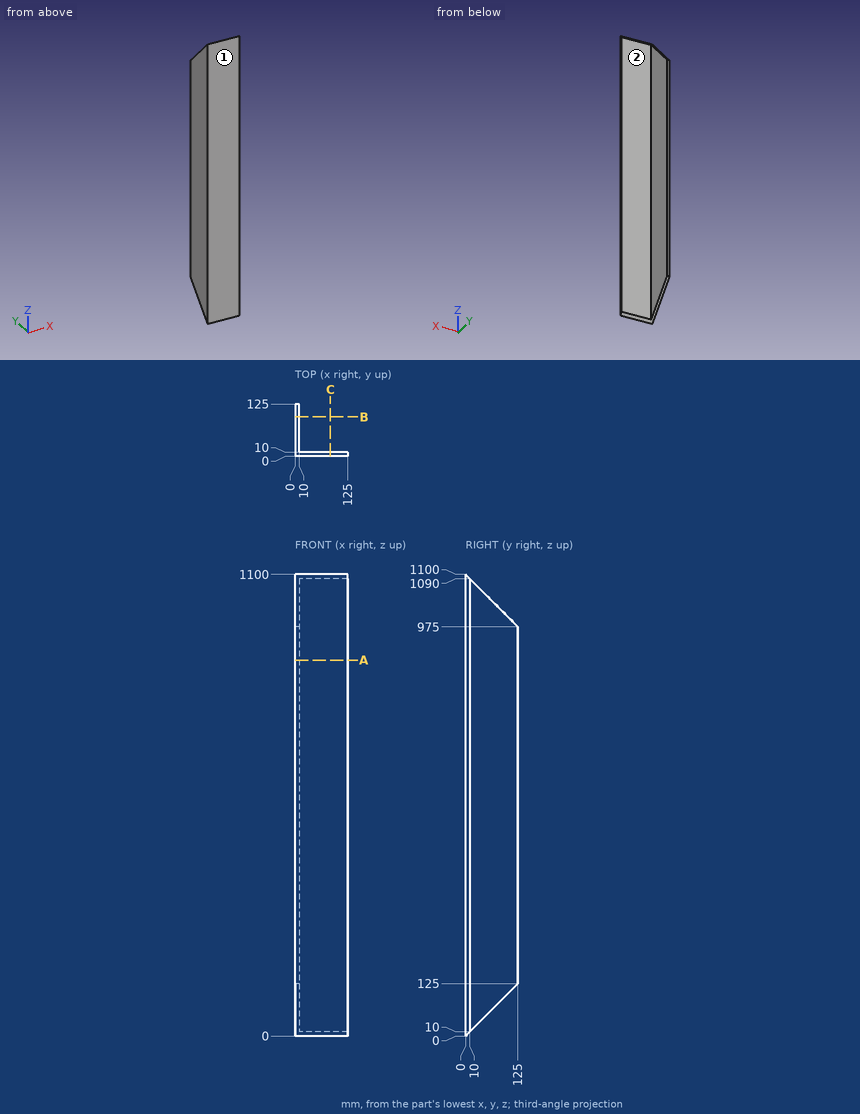
Can you work these out from the drawing? Everything is in mm from the part's minimum corner. A direction names the side the tool comes from. Coordinates: 2 decimals unless noted, no trailing zeros. Loops run counter-clockwise (first coordinate to the right, second up) from the corner with the lowest first, then second, coordinate; pieces in that order, holes last.
1) Imagine slicing it at A-A (z = 896). List the corners of the cut face in (x, y) for me.
Reported:
outline: (0, 0) - (125, 0) - (125, 10) - (10, 10) - (10, 125) - (0, 125) - close
2) Which directions (+Z, -Z, +X, -X, +Y, -Y) give clear straight access to the entire face, cutting with the end or side of a thin tool? Please do the marked faces 1 and 2.
Reported:
face 1: +Z, -Z, +X, -X, -Y
face 2: +Z, -Z, +X, +Y
3) Please list where this line runs through material, in increasing order: line 1 along Y through (x, z) = (66, 90.5).
Reported:
line 1: y = 0 to 10
4) Imagine slicing it at C-C (x = 84). List the corners of the cut face in (y, z) for me.
Reported:
outline: (0, 0) - (10, 10) - (10, 1090) - (0, 1100) - close
5) Will these pins go through, and if not, where does the flat tip stop? pin 1 Ø10 at (x, z) = (88.5, 154) entering from +Y; pin 2 Ø3 at (y, z) = (13, 331) entering from +X.
Reported:
pin 1: stops at y = 10
pin 2: stops at x = 10
6) Imagine slicing it at B-B (y = 94.5). List the corners of the cut face in (x, z) for me, and give its area (3 significant figures).
Reported:
outline: (0, 94.5) - (10, 94.5) - (10, 1005.5) - (0, 1005.5) - close
area: 9,110 mm2
